from build123d import *

# Parameters (mm, degrees)
SKETCH_1_R          = 44.5
SKETCH_1_R_2        = 32.5
EXTRUDE_1_DEPTH     = 279.1
SKETCH_2_R          = 44.5
SKETCH_2_R_2        = 43.5
CUT_EXTRUDE_1_DEPTH = 254.1
CUT_EXTRUDE_START   = -150.7
SKETCH_3_R          = 43.5
SKETCH_3_R_2        = 42.5
CUT_EXTRUDE_2_DEPTH = 150.7
CHAMFER_1_SIZE      = 2
CHAMFER_2_SIZE      = 1


with BuildPart() as part:
    # 草图1 → 凸台-拉伸1 (new body)
    with BuildSketch(Plane.XY):
        Circle(SKETCH_1_R)
        Circle(SKETCH_1_R_2, mode=Mode.SUBTRACT)
    extrude(amount=EXTRUDE_1_DEPTH)

    # 草图2 → 切除-拉伸1 (cut)
    with BuildSketch(Plane(origin=(0, 0, 25), x_dir=(-1, 0, 0), z_dir=(0, 0, -1))):
        Circle(SKETCH_2_R)
        Circle(SKETCH_2_R_2, mode=Mode.SUBTRACT)
    extrude(amount=-CUT_EXTRUDE_1_DEPTH, mode=Mode.SUBTRACT)

    # 草图3 → 切除-拉伸2 (cut)
    with BuildSketch(Plane.XY.offset(279.1).offset(CUT_EXTRUDE_START)):
        with Locations(Location((0, 0, 0), (0, 0, 180))):
            Circle(SKETCH_3_R)
        Circle(SKETCH_3_R_2, mode=Mode.SUBTRACT)
    extrude(amount=CUT_EXTRUDE_2_DEPTH, mode=Mode.SUBTRACT)

    # 倒角1
    chamfer_1_edges = [part.edges().sort_by_distance(p)[0] for p in [
        (-44.5, 0, 0),
    ]]
    chamfer(chamfer_1_edges, length=CHAMFER_1_SIZE)

    # 倒角2
    chamfer_2_edges = [part.edges().sort_by_distance(p)[0] for p in [
        (-42.5, 0, 279.1),
    ]]
    chamfer(chamfer_2_edges, length=CHAMFER_2_SIZE)


solid = part.part
Geometry check sheet. Reference: the model listing, model coordinates, mm. A direction names the side the tool comes from. Coordinates: 2 decimals unless noted, no trailing zeros. Order: outer loops, then holes, each group sorted by start corner. A loop starts at its lowest first (then second) coordinate and runs counter-clockwise, first axis right, second up. Notation, with made-up numbers: (84.5, 0) - (111.5, 0) arc R24 cw to (111.5, 28) - close; hole circle Ø9 at (80.25, -8.5). An arc over 180 degrees is marked (long way). Answer in a Markdown table with one row per item. Add a question column.
1) Cross-section at A-A, the plane y = 0. Record the cut outline in (x, z).
2) Cross-section at C-C, the plane z = 31.5. Record the cut outline in (x, y), then the cut area to 3 significant figures.
3) Material ranges on line 1 along Y through (x, z) = (0, 140); line 2 along Y through (x, z) = (0, 57); line 3 along X through (y, z) = (28, 17), recorded low to high. Write a range as [from, to].
4) Set-up check for faces 1 (the flat face through (-9.6, -31.3, 0)), 2 (the cylindrical face through (5.66, 43.13, 75.98)): record each of +Z, -Z, +X, -X, +Y, -Y from which the full face is reachable in a straight line by a thin tool's end or side.
5) Gauge pin test, flat ends, axial feed: P1, Ø4, axis at y = 6.5, z = 153.5, coming from the +X side; P2, Ø2, axis at x = 20.5, z = 242, coming from the -Y side; P3, Ø10, axis at x = -18, z = 156, coming from the +Y side. Record the tip position at first contact, or that the pin passes through.
6) Release check for a two-part mould opening along Y. For faces 3 (the cylindrical face through (31, 9.76, 137.6)), 4 (the cylindrical face through (-33.727, -25.861, 202.202)), 5 (the flat face through (-24.8, -21.3, 279.1)) record: +Y half, -Y half, draft (parallel to the pull), parting line (faces both ways), or undercut.
7) Cross-section at D-D, the plane z = 258. Record the cut outline in (x, y).
Check result:
| question | item | result |
|---|---|---|
| 1 | outline | (-44.5, 2) - (-42.5, 0) - (-32.5, 0) - (-32.5, 279.1) - (-41.5, 279.1) - (-42.5, 278.1) - (-42.5, 128.4) - (-43.5, 128.4) - (-43.5, 25) - (-44.5, 25) - close; (32.5, 0) - (42.5, 0) - (44.5, 2) - (44.5, 25) - (43.5, 25) - (43.5, 128.4) - (42.5, 128.4) - (42.5, 278.1) - (41.5, 279.1) - (32.5, 279.1) - close |
| 2 | outline | circle Ø87 at (0, 0); hole circle Ø65 at (0, 0) |
| 2 | area | 2,630 mm² |
| 3 | line 1 | y = [-42.5, -32.5], [32.5, 42.5] |
| 3 | line 2 | y = [-43.5, -32.5], [32.5, 43.5] |
| 3 | line 3 | x = [-34.59, -16.5], [16.5, 34.59] |
| 4 | face 1 | -Z, +X, -X, +Y, -Y |
| 4 | face 2 | +Z |
| 5 | P1 | stops at x = 42.26 |
| 5 | P2 | stops at y = -37.76 |
| 5 | P3 | stops at y = 40.46 |
| 6 | face 3 | undercut |
| 6 | face 4 | parting line |
| 6 | face 5 | draft |
| 7 | outline | circle Ø85 at (0, 0); hole circle Ø65 at (0, 0) |
